Source: CAD feature listing. Evaluate the final solid. Frame: model axes, mm. A direction names the side the tool comes from. Round coordinates to 2 decimals unless told otherwise and drop trailing zeros. Order: outer loops, then holes, each group sorted by start corner. A loop starts at its lowest first (then second) coordinate and runs counter-clockwise, first axis right, second up. Notation, with made-up numbers: (40.5, 42.5) -> (62.5, 42.5) arc R25 ccw to (62.5, 59.5) -> close; hole circle Ø7 at (15.25, 7.25). An arc over 180 degrees is marked (long way). Write item = value, one per line. Start each with the question number.
(1) Reachability of faces 1 (the face through (17.349, 13.957, 9.19)), 2 (the face through (-1, -30, 6)) from +Z, -Z, +X, -X, +Y, -Y: full face, straight path, thin tool, end or side. Return the list, or none.
(2) Cut plane A-A on x = 50. Return the cut outline in (y, z).
(3) Contact query for flat-ended pins moving along their axis: pin 1 Ø9 at (x, y) = (-18, -23) entering from -Z; pin 2 Ø6.5 at (x, y) = (18, 9) entering from +Z. Output: stop coordinate, or through.
(4) Cut plane C-C on x = 18. Return the cut outline in (y, z).
(5) Cut plane B-B on z = 9.75. Give the number of separate pieces and of enclosed holes in the cut face, then the cut area to 3 significant figures.
(6) Draft query along Y for faces 3 (the face through (-22, 12, 9)), 4 (the face through (-1, 30, 6)), 5 (the face through (-1, 0, 12)). Return one class per face: released by +Y, released by -Y, zero draft, split by the parting line, or undercut.
(7) Ray query, line 1 (Y direction, x = 50, z = 3.75); line 2 (Y direction, x = 18, z = 9.4); line 3 (X direction, y = -21, z = 8). Return the intervals inside material, ascending.
from build123d import *

# Parameters (mm, degrees)
SKETCH1_W                                         = 120
SKETCH1_H                                         = 60
SKETCH1_R                                         = 1.5
BOSS_EXTRUDE1_DEPTH                               = 12
HOLE_SIZE_PER_HEX_SOCKET_SCREW_TYPE_1_D           = 5.5
HOLE_SIZE_PER_HEX_SOCKET_SCREW_TYPE_1_DEPTH       = 18
HOLE_SIZE_PER_HEX_SOCKET_SCREW_TYPE_1_CBORE_D     = 10
HOLE_SIZE_PER_HEX_SOCKET_SCREW_TYPE_1_CBORE_DEPTH = 5.7
HOLE_SIZE_PER_HEX_SOCKET_SCREW_TYPE_1_TIP         = 1.652366702
M6_TAPPED_HOLE1_D                                 = 5
M6_TAPPED_HOLE1_DEPTH                             = 15
M6_TAPPED_HOLE1_TIP                               = 1.502151548


with BuildPart() as part:
    # Sketch1 → Boss-Extrude1 (new body)
    with BuildSketch(Plane.XY):
        Rectangle(SKETCH1_W, SKETCH1_H)
        with Locations((-50, 20)):
            Circle(SKETCH1_R, mode=Mode.SUBTRACT)
        with Locations((50, 20)):
            Circle(SKETCH1_R, mode=Mode.SUBTRACT)
        with Locations((50, -20)):
            Circle(SKETCH1_R, mode=Mode.SUBTRACT)
        with Locations((-50, -20)):
            Circle(SKETCH1_R, mode=Mode.SUBTRACT)
    extrude(amount=BOSS_EXTRUDE1_DEPTH)

    # Hole Size (per hex socket screw type)1
    with Locations(Plane(origin=(-18, 9, 12), x_dir=(1, 0, 0), z_dir=(0, 0, 1))):
        with Locations((0, 0), (36, 0), (0, -32), (36, -32)):
            CounterBoreHole(HOLE_SIZE_PER_HEX_SOCKET_SCREW_TYPE_1_D / 2, HOLE_SIZE_PER_HEX_SOCKET_SCREW_TYPE_1_CBORE_D / 2, HOLE_SIZE_PER_HEX_SOCKET_SCREW_TYPE_1_CBORE_DEPTH, depth=HOLE_SIZE_PER_HEX_SOCKET_SCREW_TYPE_1_DEPTH)
            with Locations((0, 0, -(HOLE_SIZE_PER_HEX_SOCKET_SCREW_TYPE_1_DEPTH + HOLE_SIZE_PER_HEX_SOCKET_SCREW_TYPE_1_TIP / 2))):  # 118° drill point
                Cone(0, HOLE_SIZE_PER_HEX_SOCKET_SCREW_TYPE_1_D / 2, HOLE_SIZE_PER_HEX_SOCKET_SCREW_TYPE_1_TIP, mode=Mode.SUBTRACT)

    # M6 Tapped Hole1
    with Locations(Plane.XY.offset(12)):
        with Locations((-50, 20), (-50, -20), (50, -20), (50, 20)):
            Hole(M6_TAPPED_HOLE1_D / 2, depth=M6_TAPPED_HOLE1_DEPTH)
            with Locations((0, 0, -(M6_TAPPED_HOLE1_DEPTH + M6_TAPPED_HOLE1_TIP / 2))):  # 118° drill point
                Cone(0, M6_TAPPED_HOLE1_D / 2, M6_TAPPED_HOLE1_TIP, mode=Mode.SUBTRACT)


solid = part.part
Evaluation:
q1.face_1 = +Z
q1.face_2 = +Z, -Z, +X, -X, -Y
q2.outline = (-30, 0) -> (-22.5, 0) -> (-22.5, 12) -> (-30, 12) -> close; (-17.5, 0) -> (17.5, 0) -> (17.5, 12) -> (-17.5, 12) -> close; (22.5, 0) -> (30, 0) -> (30, 12) -> (22.5, 12) -> close
q3.pin_1 = 0
q3.pin_2 = 6.3
q4.outline = (-30, 0) -> (-25.75, 0) -> (-25.75, 6.3) -> (-28, 6.3) -> (-28, 12) -> (-30, 12) -> close; (-20.25, 0) -> (6.25, 0) -> (6.25, 6.3) -> (4, 6.3) -> (4, 12) -> (-18, 12) -> (-18, 6.3) -> (-20.25, 6.3) -> close; (11.75, 0) -> (30, 0) -> (30, 12) -> (14, 12) -> (14, 6.3) -> (11.75, 6.3) -> close
q5.separate_pieces = 1
q5.enclosed_holes = 8
q5.area = 6,810 mm^2
q6.face_3 = undercut
q6.face_4 = released by +Y
q6.face_5 = zero draft
q7.line_1 = -30 to -22.5, -17.5 to 17.5, 22.5 to 30
q7.line_2 = -30 to -28, -18 to 4, 14 to 30
q7.line_3 = -60 to -52.29, -47.71 to -22.58, -13.42 to 13.42, 22.58 to 47.71, 52.29 to 60
